```python
from build123d import *

# Parameters (mm, degrees)
SKETCH2_OUTSIDE_W  = 14.568
SKETCH2_OUTSIDE_H  = 14.568
CUT_EXTRUDE3_DEPTH = 10
FILLET1_R          = 0.1
CHAMFER1_SIZE      = 0.5


with BuildPart() as part:
    # Sketch1 → Revolve1 (revolve)
    with BuildSketch(Plane.XY, mode=Mode.PRIVATE) as revolve1_sk:
        Polygon((0, 1), (12.5, 1), (12.5, 2.5), (7.5, 2.5), (7.5, 4.5), (6, 4.5), (6, 1.6), (3.5, 1.6), (3.5, 1.85), (2.5, 1.85), (1.5, 1.6), (0, 1.6), align=None)
    revolve(revolve1_sk.sketch.rotate(Axis((0, 0, 0), (1, 0, 0)), 90), axis=Axis((0, 0, 0), (1, 0, 0)))

    # Sketch2 outside → Cut-Extrude3 (cut)
    with BuildSketch(Plane(origin=(7.5, 0, 0), x_dir=(0, 0, -1), z_dir=(1, 0, 0))):
        Rectangle(SKETCH2_OUTSIDE_W, SKETCH2_OUTSIDE_H)
        Polygon((1.732050808, -3), (3.464101615, 0), (1.732050808, 3), (-1.732050808, 3), (-3.464101615, 0), (-1.732050808, -3), align=None, mode=Mode.SUBTRACT)
    extrude(amount=-CUT_EXTRUDE3_DEPTH, mode=Mode.SUBTRACT)

    # Fillet1
    fillet1_edges = [part.edges().sort_by_distance(p)[0] for p in [
        (0, 0, -1.6),
    ]]
    fillet(fillet1_edges, radius=FILLET1_R)

    # Chamfer1
    chamfer1_edges = [part.edges().sort_by_distance(p)[0] for p in [
        (12.5, 0, -2.5),
    ]]
    chamfer(chamfer1_edges, length=CHAMFER1_SIZE)


solid = part.part
```
CAD build for the part. Positions are in the model's coordinates, mm. A direction names the side the tool comes from. Coordinates: 2 decimals unless noted, no trailing zeros. Order: outer loops, then holes, each group sorted by start corner. A loop starts at its lowest first (then second) coordinate and runs counter-clockwise, first axis right, second up. Notation, with made-up numbers: (26, 32.5) -> (71, 32.5) arc R22 ccw to (71, 56.5) -> close; hole circle Ø7 at (69, 1). An arc over 180 degrees is marked (long way). Use one line per item in the form item = value. Start each with the question number.
1) Pull direction X, two halves, no side cores. Call faces 1 (the cylindrical face through (4.732, -0.481, 1.526)), 2 (the flat face through (7, -3, 0)), 3 (the flat face through (12.5, 1, -1)): +X half, -X half, draft (parallel to the pull), parting line (faces both ways), or undercut.
2) Drop flat-ended pins along their axis: pin 1 (4 mm diameter, centred on x = 10.5, z = -2.5, fed in from +Y); pin 2 (2 mm diameter, centred on x = 7, y = -2, fed in from -Z); pin 3 (1.5 mm diameter, centred on x = 8.5, z = -1, fed in from +Y). Give the stop position or say it passes through.
3) Band-saw the part on C-C on z = -3. Give the cut face in (x, y).
4) Band-saw the part on A-A on z = 0. Give the cut face in (x, y).
5) Drill centre lines: L1, parallel to Y at x = 10.25, z = 0; L2, parallel to Y at x = 7, z = 0; L3, parallel to X at y = 2.75, z = 0.5. Where is each one in solid material? Low to high. Write a range as [from, to].
6) Tool access for faces 4 (the cylindrical face through (0.79, -0.481, 1.526)), 5 (the flat face through (7, 3, 0)), 6 (the cylindrical face through (9.7, -0.1, -2.5)): list every direction of +Z, -Z, +X, -X, +Y, -Y with a clear straight run to the whole face (end or side of a thin tool).
7) Band-saw the part on B-B on x = 1. Give the cut face in (y, z).
Entries:
q1.face_1 = undercut
q1.face_2 = draft
q1.face_3 = +X half
q2.pin_1 = 2.45
q2.pin_2 = -2.89
q2.pin_3 = 2.49
q3.outline = (6, -0.8) -> (7.5, -0.8) -> (7.5, 0.8) -> (6, 0.8) -> close
q4.outline = (0, -1.5) arc R0.1 ccw to (0.1, -1.6) -> (1.5, -1.6) -> (2.5, -1.85) -> (3.5, -1.85) -> (3.5, -1.6) -> (6, -1.6) -> (6, -3) -> (7.5, -3) -> (7.5, -2.5) -> (12, -2.5) -> (12.5, -2) -> (12.5, -1) -> (0, -1) -> close; (0, 1) -> (12.5, 1) -> (12.5, 2) -> (12, 2.5) -> (7.5, 2.5) -> (7.5, 3) -> (6, 3) -> (6, 1.6) -> (3.5, 1.6) -> (3.5, 1.85) -> (2.5, 1.85) -> (1.5, 1.6) -> (0.1, 1.6) arc R0.1 ccw to (0, 1.5) -> close
q5.L1 = [-2.5, -1], [1, 2.5]
q5.L2 = [-3, -1], [1, 3]
q5.L3 = [6, 7.5]
q6.face_4 = -X
q6.face_5 = +Z, -Z, +X, -X, +Y
q6.face_6 = +X
q7.outline = circle Ø3.2 at (0, 0); hole circle Ø2 at (0, 0)
